Verification items for this drawing (mm, ordinates from the low corner). A direction names the side the tool comes from. Give positions to 0.01 mm unless a question says otherwise; leave off trailing zeros. Write each loop counter-clockwise with the first axis right and the second up, starting at its lowest first coordinate (ties: lowest second). Pieces come first, ordered by that corner, then holes. Notation, with made-up numbers: (38, 5.5) -> (56, 5.5) arc R11 ccw to (56, 12.5) -> close; hole circle Ø1 at (-11, 76). An arc over 180 degrees is marked (long way). Answer as a JSON object with one key per item and string values.
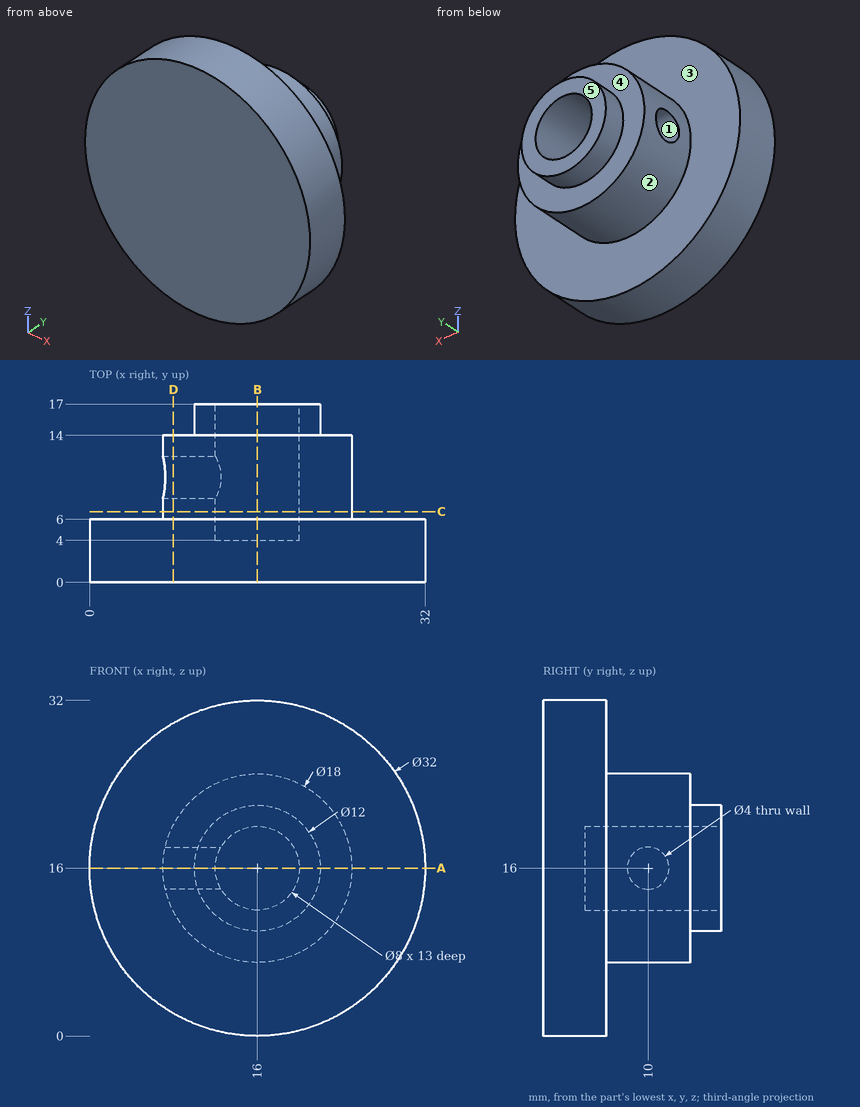
1. Sectioned sample at A-A, the plane z = 16. Enter the section's corners in (x, y), plus the area to 3 significant figures.
Determined:
{"outline": "(0, 0) -> (32, 0) -> (32, 6) -> (25, 6) -> (25, 14) -> (22, 14) -> (22, 17) -> (20, 17) -> (20, 4) -> (12, 4) -> (12, 8) -> (7, 8) -> (7, 6) -> (0, 6) -> close; (7, 12) -> (12, 12) -> (12, 17) -> (10, 17) -> (10, 14) -> (7, 14) -> close", "area": "248 mm^2"}
2. Scan lines: L1, parallel to Z at x = 16, y = 8.25; L2, parallel to X at y = 14.25, z = 16; L3, parallel to Z at x = 9.05, y = 10. Record each from-to range of solid material in increasing order. Write a range as [from, to].
Determined:
{"L1": "[7, 12], [20, 25]", "L2": "[10, 12], [20, 22]", "L3": "[10.28, 14], [18, 21.72]"}
3. Sectioned sample at D-D, the plane x = 8. Enter the section's corners in (y, z).
Determined:
{"outline": "(0, 2.14) -> (6, 2.14) -> (6, 11.88) -> (14, 11.88) -> (14, 20.12) -> (6, 20.12) -> (6, 29.86) -> (0, 29.86) -> close; hole circle Ø4 at (10, 16)"}
4. Sectioned sample at B-B, the plane x = 16. Enter the section's corners in (y, z), plus the area to 3 significant figures.
Determined:
{"outline": "(0, 0) -> (6, 0) -> (6, 7) -> (14, 7) -> (14, 10) -> (17, 10) -> (17, 12) -> (4, 12) -> (4, 20) -> (17, 20) -> (17, 22) -> (14, 22) -> (14, 25) -> (6, 25) -> (6, 32) -> (0, 32) -> close", "area": "268 mm^2"}
5. Mould release check, pull along Z, two halves, no side actions. Record for the marked faces 1, 2 and 3: released by +Z, released by -Z, zero draft, split by the parting line, or undercut.
Determined:
{"face 1": "undercut", "face 2": "split by the parting line", "face 3": "zero draft"}
6. Sectioned sample at C-C, the plane y = 6.75. Enter the section's corners in (x, z), plus the area to 3 significant figures.
Determined:
{"outline": "circle Ø18 at (16, 16); hole circle Ø8 at (16, 16)", "area": "204 mm^2"}
7. Go/stop test with flat-tipped pins: P1, Ø5, axis at x = 4, z = 12.5, coming from the +Y side; P2, Ø5, axis at y = 13.5, z = 19, coming from the +X side; P3, Ø1.5, axis at x = 25.5, y = 6, coming from the +Z side. Record where each tip stops, or that it passes through.
Determined:
{"P1": "y = 6", "P2": "x = 24.99", "P3": "z = 29.4"}
8. Access from +Z, -Z, +X, -X, +Y, -Y to the whole of each face (thin tool, end or side, straight path). Record for the marked faces 4 and 5.
Determined:
{"face 4": "+Y", "face 5": "+Z, -Z, +X, -X, +Y"}
